```python
from build123d import *

# Parameters (mm, degrees)
SKETCH1_R              = 50
BOSS_EXTRUDE1_DEPTH    = 3
SKETCH2_R              = 3.5
CUT_EXTRUDE1_DEPTH     = 71.964779997
M10X1_0_TAPPED_HOLE1_D = 9


with BuildPart() as part:
    # Sketch1 → Boss-Extrude1 (new, symmetric)
    with BuildSketch(Plane(origin=(0, 0, 0), x_dir=(1, 0, 0), z_dir=(0, 1, 0))):
        with Locations(Location((0, 0, 0), (0, 0, 270))):
            Circle(SKETCH1_R)
    extrude(amount=BOSS_EXTRUDE1_DEPTH, both=True)

    # Sketch2 → Cut-Extrude1 (cut, through all)
    with BuildSketch(Plane(origin=(0, 3, 0), x_dir=(1, 0, 0), z_dir=(0, 1, 0))):
        with Locations(Location((0, 40, 0), (0, 0, 270))):
            Circle(SKETCH2_R)
        with Locations(Location((34.641016151, -20, 0), (0, 0, 270))):
            Circle(SKETCH2_R)
        with Locations(Location((-34.641016151, -20, 0), (0, 0, 270))):
            Circle(SKETCH2_R)
    extrude(amount=-CUT_EXTRUDE1_DEPTH, mode=Mode.SUBTRACT)

    # M10x1.0 Tapped Hole1 (through all)
    with Locations(Plane(origin=(0, 3, 0), x_dir=(1, 0, 0), z_dir=(0, 1, 0))):
        with Locations((0, 0)):
            Hole(M10X1_0_TAPPED_HOLE1_D / 2)


solid = part.part
```
CAD build for the part. Positions are in the model's coordinates, mm. Coordinates: 2 decimals unless noted, no trailing zeros. Order: outer loops, then holes, each group sorted by start corner. A loop starts at its lowest first (then second) coordinate and runs counter-clockwise, first axis right, second up.
(1) Pin check, flat tips, straight feed: pin 1 Ø3 at (y, z) = (-1.5, 11.5) entering from +X; pin 2 Ø1.5 at (x, y) = (7.5, 1) entering from +Z. Stop position of each tip, or through.
Solution:
pin 1: stops at x = 48.99
pin 2: stops at z = 49.54
(2) Saw through at B-B, the plane z = 0. Write the cut outline in (x, y).
Solution:
outline: (-50, -3) - (-4.5, -3) - (-4.5, 3) - (-50, 3) - close; (4.5, -3) - (50, -3) - (50, 3) - (4.5, 3) - close
(3) Saw through at A-A, the plane x = 0. Write the cut outline in (y, z).
Solution:
outline: (-3, -50) - (3, -50) - (3, -43.5) - (-3, -43.5) - close; (-3, -36.5) - (3, -36.5) - (3, -4.5) - (-3, -4.5) - close; (-3, 4.5) - (3, 4.5) - (3, 50) - (-3, 50) - close
(4) Drill centre lines: L1, parallel to X at y = -1.5, z = 20; L2, parallel to Z at x = -3, y = -2.4; L3, parallel to Z at x = -1, y = -1.55. Where is each one in solid material? Low to high.
Solution:
L1: x = -45.83 to -38.14, -31.14 to 31.14, 38.14 to 45.83
L2: z = -49.91 to -41.8, -38.2 to -3.35, 3.35 to 49.91
L3: z = -49.99 to -43.35, -36.65 to -4.39, 4.39 to 49.99
(5) Saw through at D-D, the plane y = -0.75. Write the cut outline in (x, z).
Solution:
outline: circle Ø100 at (0, 0); hole circle Ø7 at (-34.64, 20); hole circle Ø9 at (0, 0); hole circle Ø7 at (0, -40); hole circle Ø7 at (34.64, 20)
(6) Mould opens along Z. For faces 1 (the face through (15.02, 0.04, 47.69)), 2 (the face through (0.59, -0.04, -4.46)), 3 (the face through (-10, -3, -1)) say: released by +Z, released by -Z, zero draft, split by the parting line, or undercut.
Solution:
face 1: split by the parting line
face 2: undercut
face 3: zero draft
(7) Saw through at C-C, the plane x = 36.5. Write the cut outline in (y, z).
Solution:
outline: (-3, -34.17) - (3, -34.17) - (3, 17.03) - (-3, 17.03) - close; (-3, 22.97) - (3, 22.97) - (3, 34.17) - (-3, 34.17) - close
